from build123d import *

# Parameters (mm, degrees)
EXTRUDE1_DEPTH = 45


with BuildPart() as part:
    # Sketch1 → Extrude1 (new body)
    with BuildSketch(Plane.XY):
        with BuildLine():
            Line((-23.952923538, 5.356071964), (-23.952923538, -31.593928036))
            ThreePointArc((-23.952923538, -31.593928036), (-19.896352458, -41.387356955), (-10.102923538, -45.443928036))
            Line((-10.102923538, -45.443928036), (77.647076462, -45.443928036))
            Line((77.647076462, -45.443928036), (77.647076462, -37.943928036))
            Line((77.647076462, -37.943928036), (-10.102923538, -37.943928036))
            ThreePointArc((-10.102923538, -37.943928036), (-14.593051599, -36.084056097), (-16.452923538, -31.593928036))
            Line((-16.452923538, -31.593928036), (-16.452923538, 5.356071964))
            Line((-16.452923538, 5.356071964), (-23.952923538, 5.356071964))
        make_face()
    extrude(amount=EXTRUDE1_DEPTH)


solid = part.part
Work out the finished part from the listing and answer in its coordinate system (mm). A direction names the side the tool comes from. Give positions to 0.01 mm unless a question says otherwise; leave off trailing zeros. Loops run counter-clockwise (first coordinate to the right, second up) from the corner with the lowest first, then second, coordinate; pieces in that order, holes last. Notation, with made-up numbers: (-39, 28.25) -> (10, 28.25) arc R8 ccw to (10, 32.25) -> close; hole circle Ø6 at (42.25, 26.5). An arc over 180 degrees is marked (long way). Use a Markdown table: item, result. Add a question column.
1) Consider line 1 along Y through (x, z) = (19, 9.5); line 2 along X through (y, z) = (3, 8); line 3 along X through (y, z) = (-35, 3). Determine where each line is inside the solid, lowest interval first.
2) The part is cut by section A-A, the plane z = 14.5. Determine the outline of the cut face in (x, y), plus the area to 3 significant figures.
3) The part is cut by section B-B, the plane y = -16.5. Determine the outline of the cut face in (x, z).
4) The part is cut by section C-C, the plane x = 18. Determine the outline of the cut face in (y, z), plus the area to 4 significant figures.
5) Each of these flat-tipped pins is pushed along its axis until it touches: P1, Ø5, axis at y = -8.5, z = 20, coming from the +X side; P2, Ø5, axis at y = -36, z = 27.5, coming from the -X side; P3, Ø5, axis at x = -11.5, z = 38, coming from the +Y side. Where does it stop, or does it pass through?
6) Which of the six approach directions +Z, -Z, +X, -X, +Y, -Y give full straight-line access (tool end or side, diameter ignored) to faces 1 (the flat face through (-16.453, -13, 22)), 2 (the flat face through (15, -39, 0))?
Reported:
| question | item | result |
|---|---|---|
| 1 | line 1 | y = -45.44 to -37.94 |
| 1 | line 2 | x = -23.95 to -16.45 |
| 1 | line 3 | x = -23.53 to -15.46 |
| 2 | outline | (-23.95, -31.59) arc R13.85 ccw to (-10.1, -45.44) -> (77.65, -45.44) -> (77.65, -37.94) -> (-10.1, -37.94) arc R6.35 cw to (-16.45, -31.59) -> (-16.45, 5.36) -> (-23.95, 5.36) -> close |
| 2 | area | 1,050 mm^2 |
| 3 | outline | (-23.95, 0) -> (-16.45, 0) -> (-16.45, 45) -> (-23.95, 45) -> close |
| 4 | outline | (-45.44, 0) -> (-37.94, 0) -> (-37.94, 45) -> (-45.44, 45) -> close |
| 4 | area | 337.5 mm^2 |
| 5 | P1 | stops at x = -16.45 |
| 5 | P2 | stops at x = -23.82 |
| 5 | P3 | stops at y = -36.61 |
| 6 | face 1 | +Z, -Z, +X, +Y |
| 6 | face 2 | -Z, +X, -X, +Y, -Y |
